```python
from build123d import *

# Parameters (mm, degrees)
EXTRUDE_1_DEPTH = 85
SKETCH_4_W      = 12.5
SKETCH_4_H      = 35
EXTRUDE_2_DEPTH = 45


with BuildPart() as part:
    # 草图1 → 凸台-拉伸1 (new, symmetric)
    with BuildSketch(Plane.XY):
        Polygon((0, 0), (0, 172), (14, 172), (14, 147), (12.5, 147), (12.5, 0), align=None)
    extrude(amount=EXTRUDE_1_DEPTH, both=True)

    # 草图4 → 凸台-拉伸2 (add)
    with BuildSketch(Plane(origin=(0, 0, 85), x_dir=(-1, 0, 0), z_dir=(0, 0, -1))):
        with Locations((-6.25, 126)):
            Rectangle(SKETCH_4_W, SKETCH_4_H)
    extrude(amount=-EXTRUDE_2_DEPTH)


solid = part.part
```
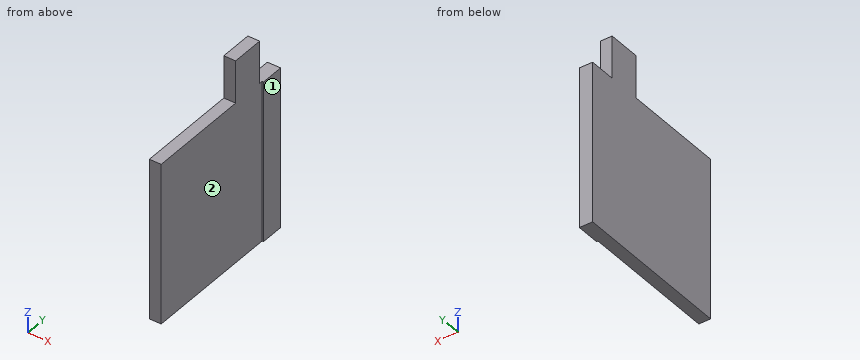
Geometry: final body of the model. Coordinates: model frame, mm. Face numbers are marked on the shaded views. A direction names the side the tool comes from. Coordinates: 2 decimals unless noted, no trailing zeros. Loops run counter-clockwise (first coordinate to the right, second up) from the corner with the lowest first, then second, coordinate; pieces in that order, holes last. Notation, with made-up numbers: M 5.5,62 L 10.5,62 A5 cw 10.5,66 Z; hole C 44.5,77 d7. An arc over 180 degrees is marked long. Put each result on its own line as item: value.
(1) Material intervals for probe 1 along Y at (x, z) = (13.75, 17); probe 2 along Z at (x, y) = (12.5, 154); probe 3 along X at (y, z) = (11.5, 33), sorted ascending.
Answer sheet:
probe 1: y = 147 to 172
probe 2: z = -85 to 85
probe 3: x = 0 to 12.5
(2) Cut plane C-C on y = 154. Return the cut outline in (x, z).
Answer sheet:
outline: M 0,-85 L 14,-85 L 14,85 L 0,85 Z
(3) Access query for the marked faces 1 and 2. Directions: +Z, -Z, +X, -X, +Y, -Y. A direction counts if a zero-diameter tool reaches every point of the face in a straight line with its end or side. Return the directions, or none.
Answer sheet:
face 1: +Z, -Z, +X, +Y, -Y
face 2: +Z, -Z, +X, -Y
(4) Cut plane B-B on x = 10. Return the cut outline in (y, z).
Answer sheet:
outline: M 0,-85 L 172,-85 L 172,85 L 143.5,85 L 143.5,130 L 108.5,130 L 108.5,85 L 0,85 Z
(5) First-contact query: pin 1 (7 mm diameter, centred on x = 4, y = 154, fed in from +Z); pin 2 (4 mm diameter, centred on x = 7.5, z = 114, fed in from -Y); pin 3 (3 mm diameter, centred on y = 122.5, z = -34, fed in from +X). Flat tips, straight axial feed; report the tip coordinate or a pass-through.
Answer sheet:
pin 1: stops at z = 85
pin 2: stops at y = 108.5
pin 3: stops at x = 12.5
(6) Cut plane D-D on y = 103.5. Return the cut outline in (x, z), then the cut area to 4 significant figures.
Answer sheet:
outline: M 0,-85 L 12.5,-85 L 12.5,85 L 0,85 Z
area: 2,125 mm^2
(7) Cut plane A-A on z = 74.5. Return the cut outline in (x, y).
Answer sheet:
outline: M 0,0 L 12.5,0 L 12.5,147 L 14,147 L 14,172 L 0,172 Z
